Read the model definition and answer for the solid it produces. Units are mm, in the model's axes. A direction names the side the tool comes from. Coordinates: 2 decimals unless noted, no trailing zeros. Write each loop counter-clockwise with the first axis right and the second up, starting at its lowest first coordinate (ties: lowest second). Pieces come first, ordered by that corner, then holes. Notation, with made-up numbers: (-27, 26.5) -> (-18, 26.5) arc R14 cw to (-18, 35.5) -> close; hole circle Ø3 at (5.25, 44). An arc over 180 degrees is marked (long way). One line per item, written item: value. Start each with the question number.
1. Consider line 1 along Y through (x, z) = (6.25, 1.05); line 2 along X through (y, z) = (-9.25, 0.2); line 3 along X through (y, z) = (-7, 1.3). Determine where each line is inside the solid, lowest interval first.
2. Find section C-C, the plane z = 0.5. Write down the section's boundary in (x, y), and give its area (3 significant figures).
3. For faces 4 (the flat face through (4.516, -10.902, 0.74)), 5 (the flat face through (4, 11, 1.5)), 6 (the cylindrical face through (-9.05, -6.73, 0.74)), determine the directions among +Z, -Z, +X, -X, +Y, -Y from which every point of the face is accessible in a straight line to the end or side of a thin tool.
4. Find section D-D, the plane x = 0. Write down the section's boundary in (y, z).
5. Find section A-A, the plane y = -4. Write down the section's boundary in (x, z), and give its area (3 significant figures).
6. Given P1, Ø1.2, axis at x = 6.3, y = -9.98, coming from the -Z side, flat-ended and moving along its own axis, determine where the tip first touches the part or whether it passes through.
7. Find section B-B, the plane x = 9.5. Write down the section's boundary in (y, z).
8. For a pull along X with two mould halves and no side action, classify faces 1 (the flat face through (-5.1, -7.4, 0.7)), 2 (the flat face through (4, 11, 0)), 3 (the cylindrical face through (-0.54, 13.94, 0.74)) as pulls with the +X half, pulls with the -X half, needs draft (parallel to the pull), parting line crosses it, or undercut.
```python
from build123d import *

# Parameters (mm, degrees)
SKETCH_1_R        = 1
EXTRUDE_952_DEPTH = 1.5


with BuildPart() as part:
    # 草图1 → Extrude 952 (new body)
    with BuildSketch(Plane.XY):
        with BuildLine():
            Line((-6.468002299, -6.001541065), (-3.669934116, -8.860004717))
            Line((-3.669934116, -8.860004717), (-5.338433881, -12.888119479))
            ThreePointArc((-5.338433881, -12.888119479), (0, 13.95), (5.338433881, -12.888119479))
            Line((5.338433881, -12.888119479), (3.669934116, -8.860004717))
            Line((3.669934116, -8.860004717), (6.468002299, -6.001541065))
            ThreePointArc((6.468002299, -6.001541065), (9.014108926, -6.738296556), (11.033790366, -5.021801727))
            ThreePointArc((11.033790366, -5.021801727), (0, 11.15), (-11.033790366, -5.021801727))
            ThreePointArc((-11.033790366, -5.021801727), (-9.014108926, -6.738296556), (-6.468002299, -6.001541065))
        make_face()
        with Locations((-6.298089329, -9.978680815)):
            Circle(SKETCH_1_R, mode=Mode.SUBTRACT)
        with Locations(Location((6.298089329, -9.978680815, 0), (0, 0, 180))):
            Circle(SKETCH_1_R, mode=Mode.SUBTRACT)
    extrude(amount=EXTRUDE_952_DEPTH)


solid = part.part
```
Answer block:
1. line 1: y = -12.47 to -10.98, -8.98 to -6.22, 9.37 to 12.47
1. line 2: x = -10.44 to -6.98, -5.61 to -3.83, 3.83 to 5.61, 6.98 to 10.44
1. line 3: x = -12.07 to -5.49, 5.49 to 12.07
2. outline: (-11.03, -5.02) arc R11.85 cw (long way) to (11.03, -5.02) arc R2.8 cw to (6.47, -6) -> (3.67, -8.86) -> (5.34, -12.89) arc R13.95 ccw (long way) to (-5.34, -12.89) -> (-3.67, -8.86) -> (-6.47, -6) arc R2.8 cw to start; hole circle Ø2 at (-6.3, -9.98); hole circle Ø2 at (6.3, -9.98)
2. area: 186 mm2
3. face 4: +Z, -Z, -Y
3. face 5: +Z, +X, -X, +Y, -Y
3. face 6: +Z, -Z
4. outline: (11.15, 0) -> (13.95, 0) -> (13.95, 1.5) -> (11.15, 1.5) -> close
5. outline: (-13.36, 0) -> (-11.38, 0) -> (-11.38, 1.5) -> (-13.36, 1.5) -> close; (11.38, 0) -> (13.36, 0) -> (13.36, 1.5) -> (11.38, 1.5) -> close
5. area: 5.95 mm2
6. P1: passes through
7. outline: (-10.22, 0) -> (-6.59, 0) -> (-6.59, 1.5) -> (-10.22, 1.5) -> close; (6.38, 0) -> (10.22, 0) -> (10.22, 1.5) -> (6.38, 1.5) -> close
8. face 1: undercut
8. face 2: needs draft
8. face 3: parting line crosses it
